from build123d import *

# Parameters (mm, degrees)
DIAMOND_PLATE_DEPTH    = 10
THROUGH_SLOTS_2X_DEPTH = 10
SLOT_BOSS_A_DEPTH      = 10
END_HOLES_PROFILE_R    = 10
END_HOLES_2X_DEPTH     = 10
SLOT_BOSS_B_DEPTH      = 10


with BuildPart() as part:
    # Diamond Plate Profile → Diamond Plate (new body)
    with BuildSketch(Plane.XY):
        with BuildLine():
            ThreePointArc((48.341000131, -83.971344784), (51.777796944, -79.503044534), (53, -74))
            Line((53, -74), (53, -44))
            ThreePointArc((53, -44), (51.777796944, -38.496955466), (48.341000131, -34.028655216))
            ThreePointArc((48.341000131, -34.028655216), (30.319444036, -14.678569552), (17.999640508, 8.718540106))
            ThreePointArc((17.999640508, 8.718540106), (0, 20), (-17.999640508, 8.718540106))
            ThreePointArc((-17.999640508, 8.718540106), (-30.319444036, -14.678569552), (-48.341000131, -34.028655216))
            ThreePointArc((-48.341000131, -34.028655216), (-51.777796944, -38.496955466), (-53, -44))
            Line((-53, -44), (-53, -74))
            ThreePointArc((-53, -74), (-51.777796944, -79.503044534), (-48.341000131, -83.971344784))
            ThreePointArc((-48.341000131, -83.971344784), (-48.2675462, -84.031821869), (-48.194149845, -84.092368816))
            ThreePointArc((-48.194149845, -84.092368816), (-30.264409293, -103.399045748), (-17.999640508, -126.718540106))
            ThreePointArc((-17.999640508, -126.718540106), (0, -138), (17.999640508, -126.718540106))
            ThreePointArc((17.999640508, -126.718540106), (30.319444036, -103.321430448), (48.341000131, -83.971344784))
        make_face()
    extrude(amount=DIAMOND_PLATE_DEPTH)

    # Slot Cuts Profile → Through Slots 2x (cut)
    with BuildSketch(Plane.XY.offset(10)):
        with BuildLine():
            Line((-47.999999999, -44), (-47.999999999, -74))
            ThreePointArc((-47.999999999, -74), (-40, -81.999999999), (-32, -74))
            Line((-32, -74), (-32, -44))
            ThreePointArc((-32, -44), (-40, -36.000000001), (-47.999999999, -44))
        make_face()
        with BuildLine():
            Line((32, -44), (32, -74))
            ThreePointArc((32, -74), (40, -81.999999999), (47.999999999, -74))
            Line((47.999999999, -74), (47.999999999, -44))
            ThreePointArc((47.999999999, -44), (40, -36.000000001), (32, -44))
        make_face()
    extrude(amount=-THROUGH_SLOTS_2X_DEPTH, mode=Mode.SUBTRACT)

    # Slot Boss A Profile → Slot Boss A (add)
    with BuildSketch(Plane.XY.offset(10)):
        with BuildLine():
            Line((-27, -44), (-27, -74))
            ThreePointArc((-27, -74), (-40, -87), (-53, -74))
            Line((-53, -74), (-53, -44))
            ThreePointArc((-53, -44), (-40, -31), (-27, -44))
        make_face()
        with BuildLine():
            Line((-32, -44), (-32, -74))
            ThreePointArc((-32, -74), (-40, -81.999999999), (-47.999999999, -74))
            Line((-47.999999999, -74), (-47.999999999, -44))
            ThreePointArc((-47.999999999, -44), (-40, -36.000000001), (-32, -44))
        make_face(mode=Mode.SUBTRACT)
    extrude(amount=SLOT_BOSS_A_DEPTH)

    # End Holes Profile → End Holes 2x (cut)
    with BuildSketch(Plane.XY.offset(10)):
        Circle(END_HOLES_PROFILE_R)
        with Locations((0, -118)):
            Circle(END_HOLES_PROFILE_R)
    extrude(amount=-END_HOLES_2X_DEPTH, mode=Mode.SUBTRACT)

    # Slot Boss B Profile → Slot Boss B (add)
    with BuildSketch(Plane.XY.offset(10)):
        with BuildLine():
            Line((27, -44), (27, -74))
            ThreePointArc((27, -74), (40, -87), (53, -74))
            Line((53, -74), (53, -44))
            ThreePointArc((53, -44), (40, -31), (27, -44))
        make_face()
        with BuildLine():
            Line((32, -44), (32, -74))
            ThreePointArc((32, -74), (40, -81.999999999), (47.999999999, -74))
            Line((47.999999999, -74), (47.999999999, -44))
            ThreePointArc((47.999999999, -44), (40, -36.000000001), (32, -44))
        make_face(mode=Mode.SUBTRACT)
    extrude(amount=SLOT_BOSS_B_DEPTH)


solid = part.part
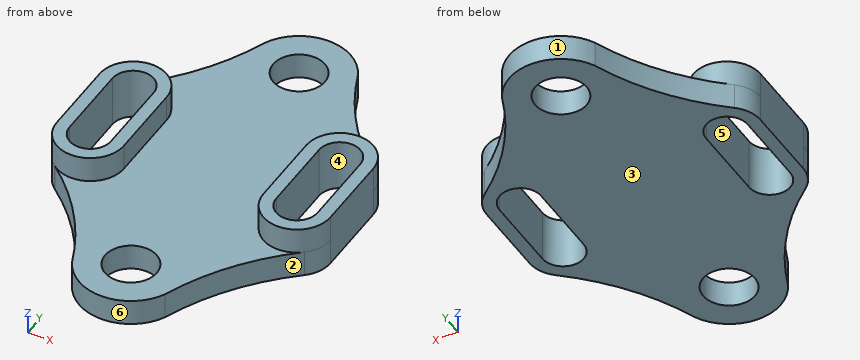
For this review, take the finished solid that the model builds, in its own axes (mm). Face numbers are marked on the shaded views. A direction names the side the tool comes from. Coordinates: 2 decimals unless noted, no trailing zeros. Loops run counter-clockwise (first coordinate to the right, second up) from the corner with the lowest first, then second, coordinate; pieces in that order, holes last. Notation, with made-up numbers: (0, 82) -> (49, 82) arc R13 cw to (49, 88) -> close; hole circle Ø7 at (-5, 55). An arc over 180 degrees is marked (long way). Write each question's results on one line, items separated by ' | '.
Q1. For pin 1 Ø4 at (x, z) = (5, 7) entering from -Y; pin 2 Ø10 at (y, z) = (-112.5, 9.5) entering from +X; pin 3 Ø12 at (x, y) = (0, -118) entering from -Z; pin 4 Ø5 at (x, y) = (17, -107) entering from +Z, all flat-tipped, find the tip position at first contact; note any pin that passes through.
Taken from the geometry:
pin 1: y = -137.77 | pin 2: x = 27.51 | pin 3: through | pin 4: z = 10
Q2. Add section B-B, the plane z = 4.75. State the section outline as (x, y) points, then the cut area to 3 significant figures.
Taken from the geometry:
outline: (-53, -74) arc R13 ccw to (-48.34, -83.97) arc R100 cw to (-48.19, -84.09) arc R100 cw to (-18, -126.72) arc R20 ccw to (18, -126.72) arc R100 cw to (48.34, -83.97) arc R13 ccw to (53, -74) -> (53, -44) arc R13 ccw to (48.34, -34.03) arc R100 cw to (18, 8.72) arc R20 ccw to (-18, 8.72) arc R100 cw to (-48.34, -34.03) arc R13 ccw to (-53, -44) -> close; hole (-48, -74) arc R8 ccw to (-32, -74) -> (-32, -44) arc R8 ccw to (-48, -44) -> close; hole circle Ø20 at (0, -118); hole circle Ø20 at (0, 0); hole (32, -74) arc R8 ccw to (48, -74) -> (48, -44) arc R8 ccw to (32, -44) -> close | area: 9,010 mm²
Q3. Machinability: for the marked faces 5 and 6, which of the approach directions +Z, -Z, +X, -X, +Y, -Y give a long, thin tool a straight path to every point of the face, cutting with its end or side? Answer none if there is none.
Taken from the geometry:
face 5: +Z, -Z | face 6: +Z, -Z, -Y
Q4. Mouldability with a two-part tool opening along X and no side actions: class the marked faces 1, 2, 3 and 4 as +X half, -X half, draft (parallel to the pull), parting line (faces both ways), or undercut.
Taken from the geometry:
face 1: parting line | face 2: +X half | face 3: draft | face 4: undercut
Q5. Add section C-C, the plane y = -118. State the section outline as (x, z) points, then the cut area to 3 significant figures.
Taken from the geometry:
outline: (-21.68, 0) -> (-10, 0) -> (-10, 10) -> (-21.68, 10) -> close; (10, 0) -> (21.68, 0) -> (21.68, 10) -> (10, 10) -> close | area: 234 mm²
Q6. Add section A-A, the plane z = 17. State the section outline as (x, y) points, then the cut area to 3 significant figures.
Taken from the geometry:
outline: (-53, -74) arc R13 ccw to (-27, -74) -> (-27, -44) arc R13 ccw to (-53, -44) -> close; (27, -74) arc R13 ccw to (53, -74) -> (53, -44) arc R13 ccw to (27, -44) -> close; hole (-48, -74) arc R8 ccw to (-32, -74) -> (-32, -44) arc R8 ccw to (-48, -44) -> close; hole (32, -74) arc R8 ccw to (48, -74) -> (48, -44) arc R8 ccw to (32, -44) -> close | area: 1,260 mm²
Q7. Add section D-D, the plane x = 40.5. State the section outline as (y, z) points.
Taken from the geometry:
outline: (-91.15, 0) -> (-81.98, 0) -> (-81.98, 20) -> (-86.99, 20) -> (-86.99, 10) -> (-91.15, 10) -> close; (-36.02, 0) -> (-26.85, 0) -> (-26.85, 10) -> (-31.01, 10) -> (-31.01, 20) -> (-36.02, 20) -> close
Q8. To check wall thickness, follow line 1 along Y through (x, z) = (0, 5.25); line 2 along X through (y, z) = (-56.5, 9.75); line 3 along X through (y, z) = (-74, 17.25). State the ranges of each line that lie inside material, in increasing order. Write a range as [from, to].
Taken from the geometry:
line 1: [-138, -128], [-108, -10], [10, 20] | line 2: [-53, -48], [-32, 32], [48, 53] | line 3: [-53, -48], [-32, -27], [27, 32], [48, 53]
